Read the model definition and answer for the solid it produces. Units are mm, in the model's axes. A direction names the side the tool comes from. Round coordinates to 2 decimals unless told otherwise and drop trailing zeros. Order: outer loops, then holes, each group sorted by start corner. A loop starts at its lowest first (then second) coordinate and runs counter-clockwise, first axis right, second up.
from build123d import *

# Parameters (mm, degrees)
SKETCH_2_R          = 1.6
CUT_EXTRUDE_1_DEPTH = 50.289958409
CUT_EXTRUDE_2_DEPTH = 50.289958409


with BuildPart() as part:
    # 草图1 → 旋转1 (revolve)
    with BuildSketch(Plane(origin=(0, 0, 0), x_dir=(1, 0, 0), z_dir=(0, 1, 0)), mode=Mode.PRIVATE) as revolve_1_sk:
        Polygon((0, 23.5), (0, 34.5), (3, 34.5), (3, 25.5), (10, 25.5), (10, 22.5), (8, 22.5), (8, 23.5), align=None)
    revolve(revolve_1_sk.sketch.rotate(Axis((-505.796489034, 0, 0), (1, 0, 0)), 180), axis=Axis((-505.796489034, 0, 0), (1, 0, 0)))

    # 草图2 → 切除-拉伸1 (cut, through all)
    with BuildSketch(Plane(origin=(3, 0, 0), x_dir=(0, 0, -1), z_dir=(1, 0, 0))):
        with Locations((0, 31.5)):
            Circle(SKETCH_2_R)
        with Locations((27.279800219, 15.75)):
            Circle(SKETCH_2_R)
        with Locations((27.279800219, -15.75)):
            Circle(SKETCH_2_R)
        with Locations((0, -31.5)):
            Circle(SKETCH_2_R)
        with Locations((-27.279800219, -15.75)):
            Circle(SKETCH_2_R)
        with Locations((-27.279800219, 15.75)):
            Circle(SKETCH_2_R)
    extrude(amount=-CUT_EXTRUDE_1_DEPTH, mode=Mode.SUBTRACT)

    # 草图3 → 切除-拉伸2 (cut, through all)
    with BuildSketch(Plane(origin=(3, 0, 0), x_dir=(0, 0, -1), z_dir=(1, 0, 0))):
        with BuildLine():
            ThreePointArc((22.627416998, 22.627416998), (16, 27.712812921), (8.282209443, 30.909626441))
            ThreePointArc((8.282209443, 30.909626441), (5.220347265, 29.141859488), (6.988114218, 26.07999731))
            ThreePointArc((6.988114218, 26.07999731), (13.5, 23.382685902), (19.091883092, 19.091883092))
            ThreePointArc((19.091883092, 19.091883092), (22.627416998, 19.091883092), (22.627416998, 22.627416998))
        make_face()
        with BuildLine():
            ThreePointArc((30.909626441, -8.282209443), (32, 0), (30.909626441, 8.282209443))
            ThreePointArc((30.909626441, 8.282209443), (27.847764263, 10.049976396), (26.07999731, 6.988114218))
            ThreePointArc((26.07999731, 6.988114218), (27, 0), (26.07999731, -6.988114218))
            ThreePointArc((26.07999731, -6.988114218), (27.847764263, -10.049976396), (30.909626441, -8.282209443))
        make_face()
        with BuildLine():
            ThreePointArc((8.282209443, -30.909626441), (16, -27.712812921), (22.627416998, -22.627416998))
            ThreePointArc((22.627416998, -22.627416998), (22.627416998, -19.091883092), (19.091883092, -19.091883092))
            ThreePointArc((19.091883092, -19.091883092), (13.5, -23.382685902), (6.988114218, -26.07999731))
            ThreePointArc((6.988114218, -26.07999731), (5.220347265, -29.141859488), (8.282209443, -30.909626441))
        make_face()
        with BuildLine():
            ThreePointArc((-22.627416998, -22.627416998), (-16, -27.712812921), (-8.282209443, -30.909626441))
            ThreePointArc((-8.282209443, -30.909626441), (-5.220347265, -29.141859488), (-6.988114218, -26.07999731))
            ThreePointArc((-6.988114218, -26.07999731), (-13.5, -23.382685902), (-19.091883092, -19.091883092))
            ThreePointArc((-19.091883092, -19.091883092), (-22.627416998, -19.091883092), (-22.627416998, -22.627416998))
        make_face()
        with BuildLine():
            ThreePointArc((-30.909626441, 8.282209443), (-32, 0), (-30.909626441, -8.282209443))
            ThreePointArc((-30.909626441, -8.282209443), (-27.847764263, -10.049976396), (-26.07999731, -6.988114218))
            ThreePointArc((-26.07999731, -6.988114218), (-27, 0), (-26.07999731, 6.988114218))
            ThreePointArc((-26.07999731, 6.988114218), (-27.847764263, 10.049976396), (-30.909626441, 8.282209443))
        make_face()
        with BuildLine():
            ThreePointArc((-8.282209443, 30.909626441), (-16, 27.712812921), (-22.627416998, 22.627416998))
            ThreePointArc((-22.627416998, 22.627416998), (-22.627416998, 19.091883092), (-19.091883092, 19.091883092))
            ThreePointArc((-19.091883092, 19.091883092), (-13.5, 23.382685902), (-6.988114218, 26.07999731))
            ThreePointArc((-6.988114218, 26.07999731), (-5.220347265, 29.141859488), (-8.282209443, 30.909626441))
        make_face()
    extrude(amount=-CUT_EXTRUDE_2_DEPTH, mode=Mode.SUBTRACT)


solid = part.part
Q1. For a pull along Y with two mould halves and no side action, classify faces 3 (the face through (10, 23, 0)), 4 (the face through (1.521, 29.195, -5.235)), 5 (the face through (6.5, 24.9, -5.5)) as released by +Y, released by -Y, zero draft, split by the parting line, or undercut.
Outcome:
face 3: zero draft
face 4: undercut
face 5: split by the parting line
Q2. A cutting plane is placed at A-A, the plane y = 0. Give the vertices of the cut face in (x, z), plus the area to 3 significant figures.
Outcome:
outline: (0, -34.5) - (3, -34.5) - (3, -32) - (0, -32) - close; (0, -27) - (3, -27) - (3, -25.5) - (10, -25.5) - (10, -22.5) - (8, -22.5) - (8, -23.5) - (0, -23.5) - close; (0, 23.5) - (8, 23.5) - (8, 22.5) - (10, 22.5) - (10, 25.5) - (3, 25.5) - (3, 27) - (0, 27) - close; (0, 32) - (3, 32) - (3, 34.5) - (0, 34.5) - close
area: 68.0 mm2
Q3. Straight lines are drawn through the part: probe 1 along Y at (x, z) = (1.85, 0); probe 2 along Y at (x, z) = (2.5, 19); probe 3 along Y at (x, z) = (6.5, 0). For each, find the intervals that lie inside material, in ascending order.
Outcome:
probe 1: y = -34.5 to -33.1, -29.9 to -23.5, 23.5 to 29.9, 33.1 to 34.5
probe 2: y = -28.8 to -25.75, -19.18 to -13.83, 13.83 to 19.18, 25.75 to 28.8
probe 3: y = -25.5 to -23.5, 23.5 to 25.5
Q4. For faces 1 (the face through (2, 0, -32)), 2 (the face through (8, 0, -23)), determine the directions among +Z, -Z, +X, -X, +Y, -Y from which every point of the face is accessible in a straight line to the end or side of a thin tool.
Outcome:
face 1: +X, -X
face 2: -X
Q5. Flat-ended cylindrical pins translate along their axes: pin 1 (23.5 mm diameter, centred on y = 6, z = -5.5, fed in from -X); pin 2 (1.5 mm diameter, centred on x = 1, y = 7.5, fed in from +Z); pin 3 (2 mm diameter, centred on x = 3, z = -17, fed in from -Y); pin 4 (3.5 mm diameter, centred on y = 15.75, z = -27.28, fed in from +X). Find the tip coordinate at first contact, or state that the pin passes through.
Outcome:
pin 1: passes through
pin 2: stops at z = 33.83
pin 3: stops at y = -30.57
pin 4: stops at x = 3
Q6. A cutting plane is placed at C-C, the plane x = 1.25. Give the number of separate pieces and of enclosed holes in the cut face, plus the area to 3 significant figures.
Outcome:
separate pieces: 1
enclosed holes: 13
area: 1,370 mm2
Q7. A cutting plane is placed at B-B, the plane z = 0. Give the vertices of the cut face in (x, y), plus the area to 3 significant figures.
Outcome:
outline: (0, -34.5) - (3, -34.5) - (3, -33.1) - (0, -33.1) - close; (0, -29.9) - (3, -29.9) - (3, -25.5) - (10, -25.5) - (10, -22.5) - (8, -22.5) - (8, -23.5) - (0, -23.5) - close; (0, 23.5) - (8, 23.5) - (8, 22.5) - (10, 22.5) - (10, 25.5) - (3, 25.5) - (3, 29.9) - (0, 29.9) - close; (0, 33.1) - (3, 33.1) - (3, 34.5) - (0, 34.5) - close
area: 78.8 mm2
